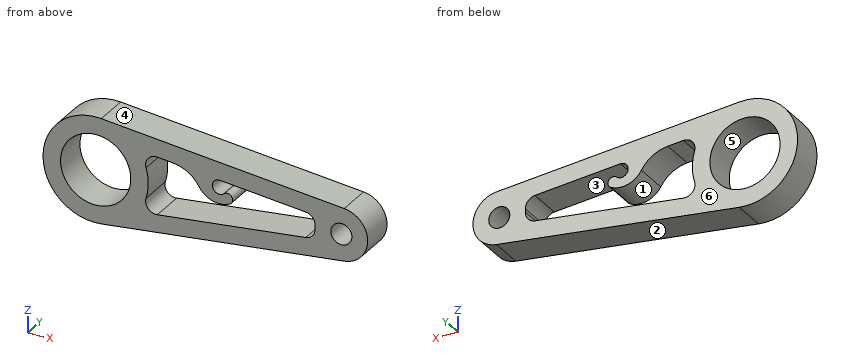
```python
from build123d import *

# Parameters (mm, degrees)
SKETCH_1_R      = 10
SKETCH_1_R_2    = 3
EXTRUDE_1_DEPTH = 10
FILLET_1_R      = 3
EXTRUDE_3_DEPTH = 10
FILLET_3_R      = 10


with BuildPart() as part:
    # 草图1 → 凸台-拉伸1 (new body)
    with BuildSketch(Plane(origin=(0, 0, 0), x_dir=(1, 0, 0), z_dir=(0, 1, 0))):
        with BuildLine():
            Line((1.607142857, 14.913654543), (70.803571429, 7.456827272))
            ThreePointArc((70.803571429, 7.456827272), (77.5, 0), (70.803571429, -7.456827272))
            Line((70.803571429, -7.456827272), (1.607142857, -14.913654543))
            ThreePointArc((1.607142857, -14.913654543), (-15, 0), (1.607142857, 14.913654543))
        make_face()
        with Locations(Location((0, 0, 0), (0, 0, 270))):
            Circle(SKETCH_1_R, mode=Mode.SUBTRACT)
        with Locations(Location((70, 0, 0), (0, 0, 270))):
            Circle(SKETCH_1_R_2, mode=Mode.SUBTRACT)
        with BuildLine():
            Line((12.187410355, 8.744542803), (63.23749297, 3.243223499))
            ThreePointArc((63.23749297, 3.243223499), (62.5, 0), (63.23749297, -3.243223499))
            Line((63.23749297, -3.243223499), (12.187410355, -8.744542803))
            ThreePointArc((12.187410355, -8.744542803), (15, 0), (12.187410355, 8.744542803))
        make_face(mode=Mode.SUBTRACT)
    extrude(amount=EXTRUDE_1_DEPTH)

    # 圆角1
    fillet_1_edges = [part.edges().sort_by_distance(p)[0] for p in [
        (12.187410355, 5, -8.744542803),
        (12.187410355, 5, 8.744542803),
        (63.23749297, 5, 3.243223499),
        (63.23749297, 5, -3.243223499),
    ]]
    fillet(fillet_1_edges, radius=FILLET_1_R)

    # 草图3 → 凸台-拉伸3 (add)
    with BuildSketch(Plane(origin=(0, 10, 0), x_dir=(1, 0, 0), z_dir=(0, 1, 0))):
        with BuildLine():
            Line((28.613097425, -6.974458511), (35.472880926, -6.235226418))
            ThreePointArc((35.472880926, -6.235226418), (33.348074169, -3.655207792), (36.559018282, -2.727232699))
            ThreePointArc((36.559018282, -2.727232699), (38.788114159, -2.411034272), (38.192669869, -0.239791316))
            ThreePointArc((38.192669869, -0.239791316), (31.413780396, -0.777770747), (28.613097425, -6.974458511))
        make_face()
    extrude(amount=-EXTRUDE_3_DEPTH)

    # 圆角3
    fillet_3_edges = [part.edges().sort_by_distance(p)[0] for p in [
        (28.613097425, 5, 6.974458511),
    ]]
    fillet(fillet_3_edges, radius=FILLET_3_R)


solid = part.part
```
Design review of the part built by this model. Coordinates are the model's own, in mm. Face numbers are marked on the shaded views. A direction names the side the tool comes from. Coordinates: 2 decimals unless noted, no trailing zeros. Order: outer loops, then holes, each group sorted by start corner. A loop starts at its lowest first (then second) coordinate and runs counter-clockwise, first axis right, second up.
1) For the marked faces 1 and 2, list the 3-axis set-ups (+Z, -Z, +X, -X, +Y, -Y) from which the entire face can be reached by the end or side of a thin tool; tool diameter is ignored.
2) Wall thickness on line 1 along Z through (x, y) = (0.5, 4.5); line 2 along Z through (x, y) = (33.5, 3.5); line 3 along Z through (x, y) = (32, 7.5): over which ranges is each line inside the solid? List them lowest first.
3) Take a section at C-C, the plane y = 1. Give the boundary of the cut face in (x, z), and give its area (3 significant figures).
4) Clearance check with flat-ended pins moving along their axes: pin 1 (1.5 mm diameter, centred on y = 8, z = -8, fed in from -X); pin 2 (4 mm diameter, centred on x = 52, y = 9, fed in from +Z); pin 3 (2 mm diameter, centred on x = 21.5, z = -9, fed in from -Y); pin 4 (1.5 mm diameter, centred on x = 59, y = 5, fed in from -Z). State where each tip first meets the part, or that it passes through.
5) Take a section at D-D, the plane x = 70. Give the boundary of the cut face in (y, z), and give its area (3 significant figures).
6) Mouldability with a two-part tool opening along X and no side actions: class the marked faces 3, 4, 5 and 6 as +X half, -X half, draft (parallel to the pull), parting line (faces both ways), or undercut.
7) Take a section at A-A, the plane x = 0. Give the boundary of the cut face in (y, z), and give its area (4 significant figures).
8) Take a section at B-B, the plane z = -5.25. Give the boundary of the cut face in (x, y), and give its area (3 significant figures).
Returned:
1. face 1: +Y, -Y
1. face 2: -Z, +X, +Y, -Y
2. line 1: z = -14.99 to -9.99, 9.99 to 14.99
2. line 2: z = -11.48 to -6.45, -0.2 to 3.29, 5.2 to 11.48
2. line 3: z = -11.64 to -6.61, 0.41 to 11.64
3. outline: (1.61, -14.91) - (70.8, -7.46) arc R7.5 ccw to (70.8, 7.46) - (1.61, 14.91) arc R15 ccw (long way) to start; hole circle Ø20 at (0, 0); hole (14.36, -4.32) arc R3 ccw to (17.56, -8.17) - (59.84, -3.61) arc R3 ccw to (62.51, -0.45) arc R7.5 cw to (62.51, 0.45) arc R3 ccw to (59.84, 3.61) - (35.47, 6.24) arc R2 ccw (long way) to (36.56, 2.73) arc R1.5 cw (long way) to (38.19, 0.24) arc R6.69 cw to (29.51, 2.84) arc R10 ccw to (21.97, 7.69) - (17.56, 8.17) arc R3 ccw to (14.36, 4.32) arc R15 cw to start; hole circle Ø6 at (70, 0)
3. area: 1,170 mm2
4. pin 1: stops at x = -13.13
4. pin 2: stops at z = 9.7
4. pin 3: stops at y = 0
4. pin 4: stops at z = -8.81
5. outline: (0, -7.54) - (10, -7.54) - (10, -3) - (0, -3) - close; (0, 3) - (10, 3) - (10, 7.54) - (0, 7.54) - close
5. area: 90.9 mm2
6. face 3: undercut
6. face 4: +X half
6. face 5: undercut
6. face 6: draft
7. outline: (0, -15) - (10, -15) - (10, -10) - (0, -10) - close; (0, 10) - (10, 10) - (10, 15) - (0, 15) - close
7. area: 100.0 mm2
8. outline: (-14.05, 0) - (-8.51, 0) - (-8.51, 10) - (-14.05, 10) - close; (8.51, 0) - (14.24, 0) - (14.24, 10) - (8.51, 10) - close; (44.62, 0) - (75.36, 0) - (75.36, 10) - (44.62, 10) - close
8. area: 420 mm2
